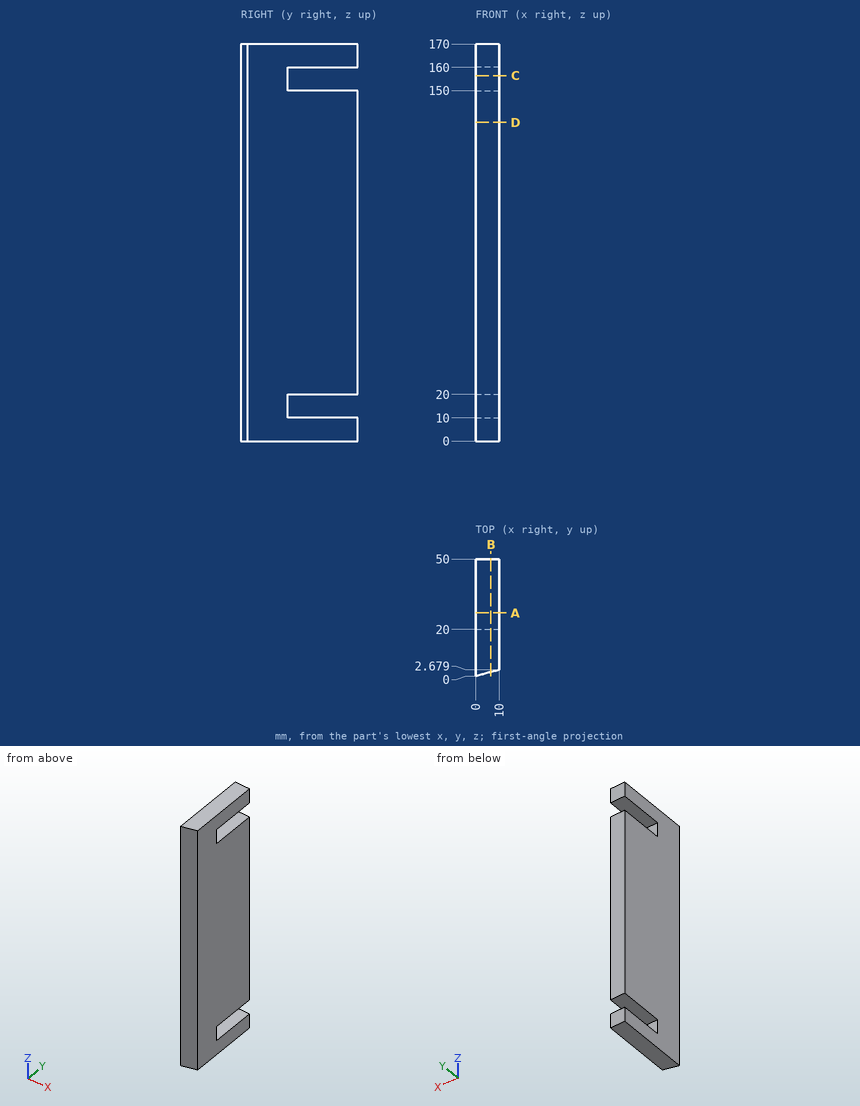
Job drawing, mm, ordinate dimensions from the low corner. One solid piece. Give positions to 0.01 mm unless a question says otherwise; leave off trailing zeros. Loops run counter-clockwise (first coordinate to the right, second up) from the corner with the lowest first, then second, coordinate; pieces in that order, holes last.
Item 1: Flat gauge pins, fed straight in: pin 1 (3 mm diameter, centred on x = 4, y = 32.5, fed in from -Z); pin 2 (3 mm diameter, centred on x = 4, z = 156.5, fed in from +Y); pin 3 (4 mm diameter, centred on x = 7, z = 77, fed in from -Y). Where does each tip first touch, or does it go through?
Answers follow:
pin 1: stops at z = 0
pin 2: stops at y = 20
pin 3: stops at y = 1.34
Item 2: Slice it at A-A, the plane y = 27. List the corners of the cut face in (x, z), and give its area (3 significant figures).
Answers follow:
outline: (0, 0) - (10, 0) - (10, 10) - (0, 10) - close; (0, 20) - (10, 20) - (10, 150) - (0, 150) - close; (0, 160) - (10, 160) - (10, 170) - (0, 170) - close
area: 1,500 mm2
Item 3: Slice it at D-D, the plane z = 136.5. List the corners of the cut face in (x, y).
Answers follow:
outline: (0, 0) - (10, 2.68) - (10, 50) - (0, 50) - close
Item 4: Drill centre lines: line 1 (Z direction, x = 5.5, y = 25.5); line 2 (Y direction, x = 5.75, z = 69.5); line 3 (Y direction, x = 9, z = 77). Where is each one in solid material? Low to high.
Answers follow:
line 1: z = 0 to 10, 20 to 150, 160 to 170
line 2: y = 1.54 to 50
line 3: y = 2.41 to 50
Item 5: Slice it at B-B, the plane x = 6.5. List the corners of the cut face in (y, z).
Answers follow:
outline: (1.74, 0) - (50, 0) - (50, 10) - (20, 10) - (20, 20) - (50, 20) - (50, 150) - (20, 150) - (20, 160) - (50, 160) - (50, 170) - (1.74, 170) - close
Item 6: Slice it at C-C, the plane z = 156.5. List the corners of the cut face in (x, y).
Answers follow:
outline: (0, 0) - (10, 2.68) - (10, 20) - (0, 20) - close
